```python
from build123d import *

# Parameters (mm, degrees)
SKETCH_1_R      = 1.55
EXTRUDE_1_DEPTH = 1.5
FILLET_1_R      = 1.5


with BuildPart() as part:
    # 草图1 → 凸台-拉伸1 (new body)
    with BuildSketch(Plane(origin=(0, 0, 0), x_dir=(1, 0, 0), z_dir=(0, 1, 0))):
        Polygon((-4, 20), (4, 20), (4, 4), (9, 4), (9, -4), (-9, -4), (-9, 4), (-4, 4), align=None)
        with Locations(Location((5, 0, 0), (0, 0, 270))):
            Circle(SKETCH_1_R, mode=Mode.SUBTRACT)
        with Locations(Location((0, 8, 0), (0, 0, 270))):
            Circle(SKETCH_1_R, mode=Mode.SUBTRACT)
        with Locations(Location((0, 16, 0), (0, 0, 270))):
            Circle(SKETCH_1_R, mode=Mode.SUBTRACT)
        with Locations(Location((-5, 0, 0), (0, 0, 90))):
            Circle(SKETCH_1_R, mode=Mode.SUBTRACT)
    extrude(amount=EXTRUDE_1_DEPTH)

    # 圆角1
    fillet_1_edges = [part.edges().sort_by_distance(p)[0] for p in [
        (4, 0.75, -4),
        (9, 0.75, -4),
        (9, 0.75, 4),
        (-9, 0.75, 4),
        (-9, 0.75, -4),
        (-4, 0.75, -4),
        (-4, 0.75, -20),
        (4, 0.75, -20),
    ]]
    fillet(fillet_1_edges, radius=FILLET_1_R)


solid = part.part
```
The listing builds one solid part. Answer for the finished solid, in the listing's coordinates (mm). A direction names the side the tool comes from. Give positions to 0.01 mm unless a question says otherwise; leave off trailing zeros. Loops run counter-clockwise (first coordinate to the right, second up) from the corner with the lowest first, then second, coordinate; pieces in that order, holes last. Notation, with made-up numbers: (-0.75, 81.5) - (4.25, 81.5) arc R23 ccw to (4.25, 95.5) - close; hole circle Ø9 at (67.25, 75). An arc over 180 degrees is marked (long way). Answer as CSV lines item,"result". Start each with the question number.
Item 1: Find the intervals of material crossed by line 1 (X direction, y = 0.65, z = 0); line 2 (X direction, y = 0.4, z = -16); line 3 (Z direction, x = 0.25, y = 0.3), in increasing order. Write a range as from..to.
Item 2: A cutting plane is placed at A-A on z = 0. Determine the outline of the cut face in (x, y).
Item 3: A cutting plane is placed at C-C on y = 0.9. Determine the outline of the cut face in (x, z), then the cut area to 3 significant figures.
Item 4: A cutting plane is placed at B-B on z = -8. Determine the outline of the cut face in (x, y).
Item 5: This flat-tipped pin is pushed along its axis until it touches: pin 1 (0.8 mm diameter, centred on y = 1, z = -10.5, fed in from -X). Where does it stop, or does it pass through?
Item 6: The mould has two halves that part along X. Classify faces 1 (the face through (-4.43, 0.76, -4.45)), 2 (the face through (0.07, 0.74, -17.55)), 3 (the face through (0, 1, -20)): +X half, -X half, draft (parallel to the pull), parting line (faces both ways), or undercut.
Item 7: For faces 4 (the face through (8.57, 0.76, 3.55)), 5 (the face through (6, 1, -4)), 6 (the face through (-4, 1, -12)), determine the directions among +Z, -Z, +X, -X, +Y, -Y from which every point of the face is accessible in a straight line to the end or side of a thin tool.
Item 8: A cutting plane is placed at D-D on x = 5. Determine the outline of the cut face in (y, z).
Found:
1,line 1,"x = -9..-6.55, -3.45..3.45, 6.55..9"
1,line 2,"x = -4..-1.55, 1.55..4"
1,line 3,"z = -20..-17.53, -14.47..-9.53, -6.47..4"
2,outline,"(-9, 0) - (-6.55, 0) - (-6.55, 1.5) - (-9, 1.5) - close; (-3.45, 0) - (3.45, 0) - (3.45, 1.5) - (-3.45, 1.5) - close; (6.55, 0) - (9, 0) - (9, 1.5) - (6.55, 1.5) - close"
3,outline,"(-9, -2.5) arc R1.5 ccw to (-7.5, -4) - (-5.5, -4) arc R1.5 cw to (-4, -5.5) - (-4, -18.5) arc R1.5 ccw to (-2.5, -20) - (2.5, -20) arc R1.5 ccw to (4, -18.5) - (4, -5.5) arc R1.5 cw to (5.5, -4) - (7.5, -4) arc R1.5 ccw to (9, -2.5) - (9, 2.5) arc R1.5 ccw to (7.5, 4) - (-7.5, 4) arc R1.5 ccw to (-9, 2.5) - close; hole circle Ø3.1 at (-5, 0); hole circle Ø3.1 at (0, -16); hole circle Ø3.1 at (0, -8); hole circle Ø3.1 at (5, 0)"
3,area,"240 mm^2"
4,outline,"(-4, 0) - (-1.55, 0) - (-1.55, 1.5) - (-4, 1.5) - close; (1.55, 0) - (4, 0) - (4, 1.5) - (1.55, 1.5) - close"
5,pin 1,"stops at x = -4"
6,face 1,"-X half"
6,face 2,"undercut"
6,face 3,"draft"
7,face 4,"+Z, +X, +Y, -Y"
7,face 5,"-Z, +X, +Y, -Y"
7,face 6,"-Z, -X, +Y, -Y"
8,outline,"(0, -4.09) - (1.5, -4.09) - (1.5, -1.55) - (0, -1.55) - close; (0, 1.55) - (1.5, 1.55) - (1.5, 4) - (0, 4) - close"
